from build123d import *

# Parameters (mm, degrees)
SKETCH_1_W                  = 25
SKETCH_1_H                  = 62
EXTRUDE_1_DEPTH             = 8
SKETCH_2_W                  = 133.5
SKETCH_2_H                  = 5
PATTERN_LINEAR_1_COUNT      = 2
PATTERN_LINEAR_1_PITCH      = 38
PATTERN_LINEAR_2_COUNT      = 2
PATTERN_LINEAR_2_PITCH      = 16
PATTERN_LINEAR_2_COUNT_DIR2 = 2
PATTERN_LINEAR_2_PITCH_DIR2 = 52


with BuildPart() as part:
    # 草图1 → 凸台-拉伸1 (new body)
    with BuildSketch(Plane(origin=(0, 0, 0), x_dir=(0, 0, -1), z_dir=(1, 0, 0))):
        Rectangle(SKETCH_1_W, SKETCH_1_H)
    extrude(amount=-EXTRUDE_1_DEPTH)

    # 草图2 → 旋转1 (revolve)
    with BuildSketch(Plane.XY, mode=Mode.PRIVATE) as revolve_1_sk:
        with Locations((66.75, 21.5)):
            Rectangle(SKETCH_2_W, SKETCH_2_H)
    revolve_1 = revolve(revolve_1_sk.sketch.rotate(Axis((133.5, 19, 0), (-1, 0, 0)), 270), axis=Axis((133.5, 19, 0), (-1, 0, 0)))

    # 阵列(线性)1: 旋转1 ×2
    with Locations(*[(0, -i * PATTERN_LINEAR_1_PITCH, 0) for i in range(1, PATTERN_LINEAR_1_COUNT)]):
        add(revolve_1)

    # 草图4 → 切除-旋转1 (revolve, cut)
    with BuildSketch(Plane.XY.offset(8), mode=Mode.PRIVATE) as cut_revolve_1_sk:
        Polygon((-8, 26), (-8, 28.5), (-7.567, 28.067), (-0.433, 28.067), (0, 28.5), (0, 26), align=None)
    cut_revolve_1 = revolve(cut_revolve_1_sk.sketch.rotate(Axis((0, 26, 8), (-1, 0, 0)), 270), axis=Axis((0, 26, 8), (-1, 0, 0)), mode=Mode.SUBTRACT)

    # 阵列(线性)2: Cut-Revolve 1 2 × 2
    with Locations(*[(0, -j * PATTERN_LINEAR_2_PITCH_DIR2, -i * PATTERN_LINEAR_2_PITCH) for i in range(PATTERN_LINEAR_2_COUNT) for j in range(PATTERN_LINEAR_2_COUNT_DIR2) if (i, j) != (0, 0)]):
        add(cut_revolve_1, mode=Mode.SUBTRACT)

    # 草图6 → 旋转2 (revolve)
    with BuildSketch(Plane.XY, mode=Mode.PRIVATE) as revolve_2_sk:
        Polygon((0, 0), (0, 4), (118.5, 4), (118.5, 8), (123.5, 8), (123.5, 0), align=None)
    revolve(revolve_2_sk.sketch.rotate(Axis((123.5, 0, 0), (-1, 0, 0)), 270), axis=Axis((123.5, 0, 0), (-1, 0, 0)))


solid = part.part
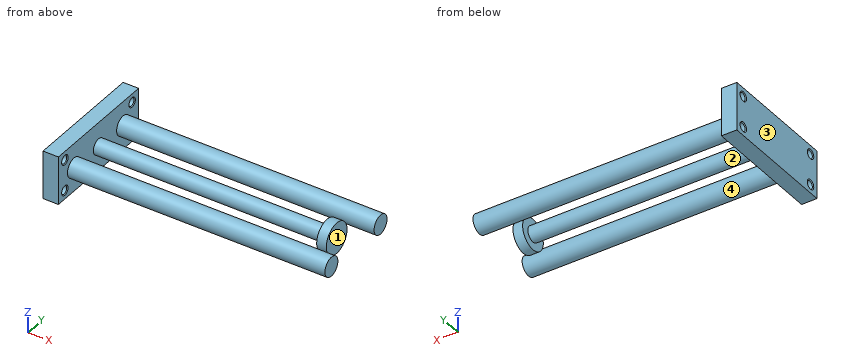
Geometry check sheet. Reference: the model listing, model coordinates, mm. Face numbers are marked on the shaded views. Round coordinates to 2 decimals unless told otherwise and drop trailing zeros. Loops run counter-clockwise (first coordinate to the right, second up) from the corner with the lowest first, then second, coordinate; pieces in that order, holes last. Notation, with made-up numbers: (62, 44.25) - (104, 44.25) arc R18 ccw to (104, 78.25) - close; hole circle Ø9 at (-3.75, -8). An arc over 180 degrees is marked (long way). One line per question, with ' | ' between items. Start each with the question number.
1. Depth check by flat-ended pin: pin 1 (4 mm diameter, centred on x = 73, z = -6.5, fed in from +Y); pin 2 (2 mm diameter, centred on x = 92, y = 16, fed in from -Z); pin 3 (5 mm diameter, centred on x = 110.5, z = -5, fed in from -Y); pin 4 (6.5 mm diameter, centred on y = -26, z = 8, fed in from -X). Enter the tip coordinate at first touch or a pass-through.
2. Cross-section at C-C on x = 1.5. Record the cut outline in (y, z), then the cut area to 3 significant figures.
3. Scan lines: line 1 (Y direction, x = -3, z = -8); line 2 (Y direction, x = 41.5, z = 0.5); line 3 (X direction, y = 0.5, z = -6.5). Record each from-to range of solid material in increasing order. Write a range as [from, to].
4. Cross-section at A-A on y = -26. Record the cut outline in (x, z), then the cut area to 3 significant figures.
5. Cross-section at D-D on z = 0.5. Record the cut outline in (x, y).
6. Cross-section at B-B on y = 0. Record the cut outline in (x, z).
7. Draft check along X on the marked faces 1, 2, 3 and 4. Enter one of: released by +X, released by -X, zero draft, split by the parting line, or undercut.
Taken from the geometry:
1) pin 1: y = 21.18 | pin 2: z = -4.58 | pin 3: y = -23.33 | pin 4: x = -8
2) outline: circle Ø10 at (-19, 0); circle Ø8 at (0, 0); circle Ø10 at (19, 0) | area: 207 mm²
3) line 1: [-31, -28.07], [-23.93, 23.93], [28.07, 31] | line 2: [-23.97, -14.03], [-3.97, 3.97], [14.03, 23.97] | line 3: [-8, 0], [118.5, 123.5]
4) outline: (-8, -12.5) - (0, -12.5) - (0, -10.5) - (-0.43, -10.07) - (-7.57, -10.07) - (-8, -10.5) - close; (-8, -5.5) - (-7.57, -5.93) - (-0.43, -5.93) - (0, -5.5) - (0, 5.5) - (-0.43, 5.93) - (-7.57, 5.93) - (-8, 5.5) - close; (-8, 10.5) - (-7.57, 10.07) - (-0.43, 10.07) - (0, 10.5) - (0, 12.5) - (-8, 12.5) - close | area: 133 mm²
5) outline: (-8, -31) - (0, -31) - (0, -23.97) - (133.5, -23.97) - (133.5, -14.03) - (0, -14.03) - (0, -3.97) - (118.5, -3.97) - (118.5, -7.98) - (123.5, -7.98) - (123.5, 7.98) - (118.5, 7.98) - (118.5, 3.97) - (0, 3.97) - (0, 14.03) - (133.5, 14.03) - (133.5, 23.97) - (0, 23.97) - (0, 31) - (-8, 31) - close
6) outline: (-8, -12.5) - (0, -12.5) - (0, -4) - (118.5, -4) - (118.5, -8) - (123.5, -8) - (123.5, 8) - (118.5, 8) - (118.5, 4) - (0, 4) - (0, 12.5) - (-8, 12.5) - close
7) face 1: released by +X | face 2: undercut | face 3: released by -X | face 4: zero draft
